from build123d import *

# Parameters (mm, degrees)
BOSS_EXTRUDE1_DEPTH = 1063.8155
CUT_EXTRUDE1_DEPTH  = 150
SKETCH3_R           = 7.14375
CUT_EXTRUDE2_DEPTH  = 250


with BuildPart() as part:
    # Sketch1 → Boss-Extrude1 (new, symmetric)
    with BuildSketch(Plane.XY):
        Polygon((0, 127), (0, 0), (127, 0), (127, 7.9375), (7.9375, 7.9375), (7.9375, 127), align=None)
    extrude(amount=BOSS_EXTRUDE1_DEPTH, both=True)

    # Sketch2 → Cut-Extrude1 (cut)
    with BuildSketch(Plane.ZY):
        Polygon((1063.8155, 0), (1042.676904036, 127), (1063.8155, 127), align=None)
    extrude(amount=-CUT_EXTRUDE1_DEPTH, mode=Mode.SUBTRACT)

    # Sketch3 → Cut-Extrude2 (cut, symmetric)
    with BuildSketch(Plane(origin=(0, 7.9375, 0), x_dir=(1, 0, 0), z_dir=(0, 1, 0))):
        with Locations(Location((88.9, -879.2845, 0), (0, 0, 270))):
            Circle(SKETCH3_R)
        Polygon((0, -1063.8155), (127, -1063.8155), (127, -1045.559770079), align=None)
        with BuildLine():
            Line((70.64375, 916.97175), (70.64375, 880.45925))
            ThreePointArc((70.64375, 880.45925), (63.5, 873.3155), (56.35625, 880.45925))
            Line((56.35625, 880.45925), (56.35625, 916.97175))
            ThreePointArc((56.35625, 916.97175), (63.5, 924.1155), (70.64375, 916.97175))
        make_face()
    extrude(amount=CUT_EXTRUDE2_DEPTH, both=True, mode=Mode.SUBTRACT)


solid = part.part
Part model, mm, in its own coordinate system. A direction names the side the tool comes from. Coordinates: 2 decimals unless noted, no trailing zeros. Loops run counter-clockwise (first coordinate to the right, second up) from the corner with the lowest first, then second, coordinate; pieces in that order, holes last. Notation, with made-up numbers: (6.5, 52.5) - (54.5, 52.5) arc R20 cw to (54.5, 82.5) - close; hole circle Ø5 at (83, 40). An arc over 180 degrees is marked (long way). Write each question's results on one line, items separated by ' | '. Start each with the question number.
Q1. Drop flat-ended pins along their axis: pin 1 Ø3 at (y, z) = (44.5, -247) entering from -X; pin 2 Ø2 at (y, z) = (22, 29.5) entering from +X; pin 3 Ø1 at (x, z) = (92.5, 612) entering from +Y; pin 4 Ø8.5 at (x, z) = (88.9, 879.28) entering from -Y. Give the stop position or say it passes through.
Q2. Probe line 1 along X through (y, z) = (107.5, -209); line 2 along Z through (x, y) = (88, 2). List the from-to ranges inside material, lowest first.
Q3. Slice it at A-A on z = 158. Give the cut face in (x, y).
Q4. Which spindle directions (+Z, -Z, +X, -X, +Y, -Y) get a long thin tool onto all of the face, cutting with end or side? Do faces 1 (the flat face through (7.938, 67, 14)), 2 (the flat face through (7, 36, -1063.816)). Say none if no direction does.
Q5. Slice it at B-B on x = 32.5. Give the cut face in (y, z), and give its area (3 significant figures).
Q6. Slice it at C-C on y = 65. Give the cut face in (x, z).
Answer:
1) pin 1: stops at x = 0 | pin 2: stops at x = 7.94 | pin 3: stops at y = 7.94 | pin 4: passes through
2) line 1: x = 0 to 7.94 | line 2: z = -1063.82 to 872.2, 886.37 to 1051.17
3) outline: (0, 0) - (127, 0) - (127, 7.94) - (7.94, 7.94) - (7.94, 127) - (0, 127) - close
4) face 1: +Z, -Z, +X, +Y | face 2: -Z, +X, -X, +Y, -Y
5) outline: (0, -1063.82) - (7.94, -1063.82) - (7.94, 1059.14) - (0, 1059.14) - close | area: 16,900 mm2
6) outline: (0, -1063.82) - (7.94, -1063.82) - (7.94, 1053) - (0, 1053) - close
